Verification items for the finished model (mm, model axes). A direction names the side the tool comes from. Coordinates: 2 decimals unless noted, no trailing zeros. Loops run counter-clockwise (first coordinate to the right, second up) from the corner with the lowest first, then second, coordinate; pieces in that order, holes last. Notation, with made-up numbers: (29.25, 2) -> (65.25, 2) arc R23 cw to (65.25, 23) -> close; hole circle Ø6 at (-18, 41). An arc over 180 degrees is marked (long way). Write item = value, one per line.
```python
from build123d import *

# Parameters (mm, degrees)
SKETCH_1_R      = 25
EXTRUDE_1_DEPTH = 10
SKETCH_2_R      = 8
EXTRUDE_2_DEPTH = 60
CHAMFER_1_SIZE  = 1


with BuildPart() as part:
    # 草图1 → 凸台-拉伸1 (new body)
    with BuildSketch(Plane(origin=(0, 0, 0), x_dir=(0, 0, -1), z_dir=(1, 0, 0))):
        Circle(SKETCH_1_R)
    extrude(amount=EXTRUDE_1_DEPTH)

    # 草图2 → 凸台-拉伸2 (add)
    with BuildSketch(Plane(origin=(10, 0, 0), x_dir=(0, 0, -1), z_dir=(1, 0, 0))):
        Circle(SKETCH_2_R)
    extrude(amount=EXTRUDE_2_DEPTH)

    # 草图3 → 旋转1 (revolve)
    with BuildSketch(Plane.XY, mode=Mode.PRIVATE) as revolve_1_sk:
        Polygon((70, 8), (86, 0), (70, 0), align=None)
    revolve(revolve_1_sk.sketch.rotate(Axis((0, 0, 0), (1, 0, 0)), 90), axis=Axis((0, 0, 0), (1, 0, 0)))

    # 倒角1
    chamfer_1_edges = [part.edges().sort_by_distance(p)[0] for p in [
        (0, 0, 25),
        (10, 0, 25),
    ]]
    chamfer(chamfer_1_edges, length=CHAMFER_1_SIZE)


solid = part.part
```
1) Sectioned sample at B-B, the plane x = 53. Record the cut outline in (y, z).
Ans:
outline = circle Ø16 at (0, 0)
2) Depth check by flat-ended pin: pin 1 Ø10 at (y, z) = (-0.5, -20) entering from +X; pin 2 Ø3 at (x, y) = (14, 6) entering from +Z; pin 3 Ø12 at (x, y) = (17, 12.5) entering from +Z. Enter the tip coordinate at first touch or a pass-through.
Ans:
pin_1 = 10
pin_2 = 6.61
pin_3 = 4.66
3) Release check for a two-part mould opening along Y. For faces 3 (the face through (39.58, -7.81, 1.73)), 4 (the face through (0, 0, 0)) record: pulls with the +Y half, pulls with the -Y half, needs draft (parallel to the pull), parting line crosses it, or undercut.
Ans:
face_3 = parting line crosses it
face_4 = needs draft
4) Sectioned sample at A-A, the plane x = 80. Record the cut outline in (y, z), plus the area to 3 significant figures.
Ans:
outline = circle Ø6 at (0, 0)
area = 28.3 mm2
5) Tool access check on faces 1 (the face through (10, 6, 6)), 2 (the face through (4.944, 7.509, -23.846)). Record the directions out of +Z, -Z, +X, -X, +Y, -Y that give a thin tool (end or side, any length) a straight path to the whole face; none if there is none.
Ans:
face_1 = +X
face_2 = +X, -X
6) Material ranges on line 1 (X direction, y = -20.5, z = -10.5); line 2 (Z direction, x = 19.5, y = 5) (3 decimals); line 3 (Z direction, x = 20, y = -6), recorded low to high.
Ans:
line_1 = 0 to 10
line_2 = -6.245 to 6.245
line_3 = -5.29 to 5.29
